Input: dimensioned drawing with shaded views. Units: mm. Origin: part minimum x, y, z. A direction names the side the tool comes from. Round coordinates to 2 decimals unless told otherwise and drop trailing zeros. Loops run counter-clockwise (first coordinate to the right, second up) from the corner with the lowest first, then second, coordinate; pieces in that order, holes last. Notation, with made-up numbers: M 76.25,-1 L 121.25,-1 A8 cw 121.25,9 Z; hole C 55,46 d2. An arc over 180 degrees is marked long. One line per item, written item: value.
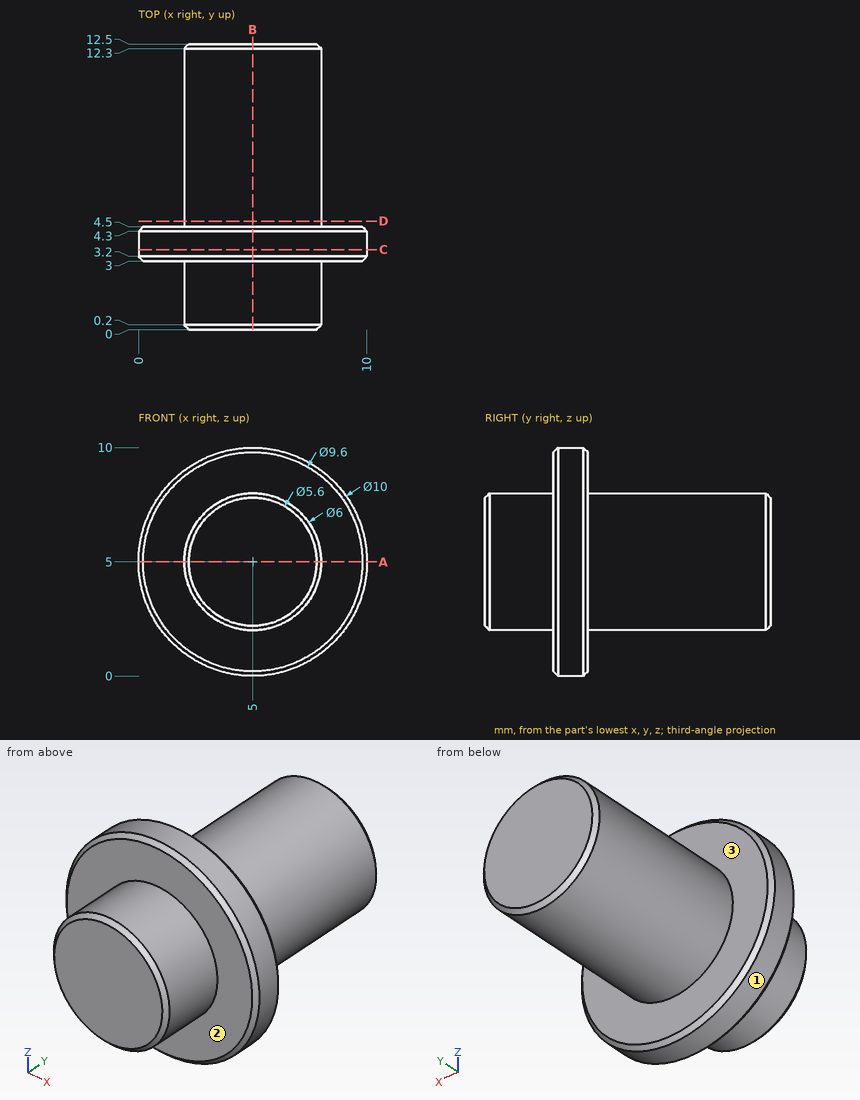
1. Reachability of the marked faces 1, 2 and 3 from +Z, -Z, +X, -X, +Y, -Y: full face, straight path, thin tool, end or side. Return the list, or none.
Report:
face 1: +Y, -Y
face 2: -Y
face 3: +Y
2. Section query A-A (z = 5). Return the cut outline in (x, y), and give its area (3 significant figures).
Report:
outline: M 0,3.2 L 0.2,3 L 2,3 L 2,0.2 L 2.2,0 L 7.8,0 L 8,0.2 L 8,3 L 9.8,3 L 10,3.2 L 10,4.3 L 9.8,4.5 L 8,4.5 L 8,12.3 L 7.8,12.5 L 2.2,12.5 L 2,12.3 L 2,4.5 L 0.2,4.5 L 0,4.3 Z
area: 80.8 mm2
3. Ray query, line 1 (Y direction, x = 8, z = 7); line 2 (Z direction, x = 4.5, y = 2); line 3 (X direction, y = 3.5, z = 2.25). Return the intervals inside material, ascending. Write a range as [from, to].
Report:
line 1: y = [3, 4.5]
line 2: z = [2.04, 7.96]
line 3: x = [0.82, 9.18]
4. Section query C-C (y = 3.5). Return the cut outline in (x, z), and give its area (3 significant figures).
Report:
outline: C 5,5 d10
area: 78.5 mm2
5. Section query B-B (x = 5). Return the cut outline in (y, z).
Report:
outline: M 0,2.2 L 0.2,2 L 3,2 L 3,0.2 L 3.2,0 L 4.3,0 L 4.5,0.2 L 4.5,2 L 12.3,2 L 12.5,2.2 L 12.5,7.8 L 12.3,8 L 4.5,8 L 4.5,9.8 L 4.3,10 L 3.2,10 L 3,9.8 L 3,8 L 0.2,8 L 0,7.8 Z
6. Pin query (flat end, axial travel): pin 1 (5 mm diameter, centred on x = 8.5, z = 6, fed in from +Y); pin 2 (1 mm diameter, centred on x = 8, y = 11, fed in from +Z). Return the tip coordinate at first contact, or that it passes through.
Report:
pin 1: stops at y = 12.5
pin 2: stops at z = 6.66
7. Section query D-D (y = 4.75). Return the cut outline in (x, z), and give its area (3 significant figures).
Report:
outline: C 5,5 d6
area: 28.3 mm2
